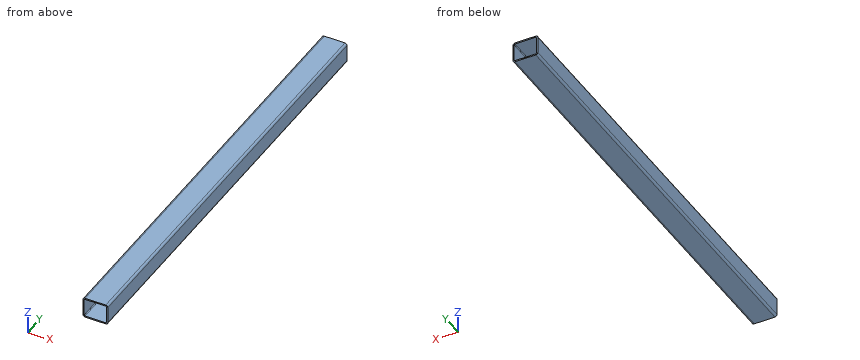
from build123d import *

# Parameters (mm, degrees)
EXTRUDE_THIN1_DEPTH = 1057


with BuildPart() as part:
    # Sketch1 → Extrude-Thin1 (new, symmetric)
    with BuildSketch(Plane(origin=(0, 0, 0), x_dir=(1, 0, 0), z_dir=(0, 1, 0))):
        with BuildLine():
            Line((-50, 50), (50, 50))
            ThreePointArc((50, 50), (57.071067812, 47.071067812), (60, 40))
            Line((60, 40), (60, -40))
            ThreePointArc((60, -40), (57.071067812, -47.071067812), (50, -50))
            Line((50, -50), (-50, -50))
            ThreePointArc((-50, -50), (-57.071067812, -47.071067812), (-60, -40))
            Line((-60, -40), (-60, 40))
            ThreePointArc((-60, 40), (-57.071067812, 47.071067812), (-50, 50))
        make_face()
        with BuildLine():
            Line((-50, 44), (50, 44))
            ThreePointArc((50, 44), (52.828427125, 42.828427125), (54, 40))
            Line((54, 40), (54, -40))
            ThreePointArc((54, -40), (52.828427125, -42.828427125), (50, -44))
            Line((50, -44), (-50, -44))
            ThreePointArc((-50, -44), (-52.828427125, -42.828427125), (-54, -40))
            Line((-54, -40), (-54, 40))
            ThreePointArc((-54, 40), (-52.828427125, 42.828427125), (-50, 44))
        make_face(mode=Mode.SUBTRACT)
    extrude(amount=EXTRUDE_THIN1_DEPTH, both=True)


solid = part.part
Build history of the part. All positions in model axes, mm. Round coordinates to 2 decimals unless told otherwise and drop trailing zeros. Loops run counter-clockwise (first coordinate to the right, second up) from the corner with the lowest first, then second, coordinate; pieces in that order, holes last. Notation, with made-up numbers: (-30.5, -23) -> (23.5, -23) arc R22 ccw to (23.5, 2) -> close; hole circle Ø8 at (29.5, 16). An arc over 180 degrees is marked (long way). Answer in a Markdown table with one row per item.
Item 1: Saw through at C-C (y = -724). Write the cut outline in (x, z).
Answers below:
| item | result |
|---|---|
| outline | (-60, -40) arc R10 ccw to (-50, -50) -> (50, -50) arc R10 ccw to (60, -40) -> (60, 40) arc R10 ccw to (50, 50) -> (-50, 50) arc R10 ccw to (-60, 40) -> close; hole (-54, -40) arc R4 ccw to (-50, -44) -> (50, -44) arc R4 ccw to (54, -40) -> (54, 40) arc R4 ccw to (50, 44) -> (-50, 44) arc R4 ccw to (-54, 40) -> close |
Item 2: Saw through at A-A (z = -13.5). Write the cut outline in (x, y).
Answers below:
| item | result |
|---|---|
| outline | (-60, -1057) -> (-54, -1057) -> (-54, 1057) -> (-60, 1057) -> close; (54, -1057) -> (60, -1057) -> (60, 1057) -> (54, 1057) -> close |
Item 3: Saw through at B-B (x = -11). Write the cut outline in (y, z), and give its area (3 significant figures).
Answers below:
| item | result |
|---|---|
| outline | (-1057, -50) -> (1057, -50) -> (1057, -44) -> (-1057, -44) -> close; (-1057, 44) -> (1057, 44) -> (1057, 50) -> (-1057, 50) -> close |
| area | 25,400 mm² |
Item 4: Drill centre lines: L1, parallel to Z at x = 1, y = 211.5; L2, parallel to X at y = 739.5, z = -4.5; L3, parallel to X at y = -100.5, z = -45. Where is each one in solid material? Low to high. Write a range as [from, to].
Answers below:
| item | result |
|---|---|
| L1 | z = [-50, -44], [44, 50] |
| L2 | x = [-60, -54], [54, 60] |
| L3 | x = [-58.66, 58.66] |
